Geometry: final body of the model. Coordinates: model frame, mm. Coordinates: 2 decimals unless noted, no trailing zeros. Order: outer loops, then holes, each group sorted by start corner. A loop starts at its lowest first (then second) coordinate and runs counter-clockwise, first axis right, second up. Notation, with made-up numbers: (64, -35.75) - (110, -35.75) arc R17 cw to (110, -16.75) - close; hole circle Ø8 at (-17, -18.5). An arc over 180 degrees is marked (long way). Use a Markdown table: item, result. Add a question column.
```python
from build123d import *

# Parameters (mm, degrees)
SKETCH_1_R          = 37.5
SKETCH_1_R_2        = 32.5
EXTRUDE_1_DEPTH     = 50
SKETCH_2_R          = 92.5
SKETCH_2_R_2        = 37.5
SKETCH_2_R_3        = 9
EXTRUDE_2_DEPTH     = 20
SKETCH_3_R          = 37.5
EXTRUDE_3_DEPTH     = 20
SKETCH_4_R          = 32.5
CUT_EXTRUDE_1_DEPTH = 141.044635742


with BuildPart() as part:
    # Sketch 1 → Extrude 1 (new body)
    with BuildSketch(Plane(origin=(0, 0, 0), x_dir=(1, 0, 0), z_dir=(0, 1, 0))):
        with Locations(Location((0, 0, 0), (0, 0, 270))):
            Circle(SKETCH_1_R)
        with Locations(Location((0, 0, 0), (0, 0, 270))):
            Circle(SKETCH_1_R_2, mode=Mode.SUBTRACT)
    extrude(amount=EXTRUDE_1_DEPTH)



with BuildPart() as body_2:
    # Sketch 2 → Extrude 2 (new body)
    with BuildSketch(Plane(origin=(0, 50, 0), x_dir=(1, 0, 0), z_dir=(0, 1, 0))):
        with Locations(Location((0, 0, 0), (0, 0, 270))):
            Circle(SKETCH_2_R)
        with Locations(Location((0, 0, 0), (0, 0, 270))):
            Circle(SKETCH_2_R_2, mode=Mode.SUBTRACT)
        with Locations(Location((-72.5, 0, 0), (0, 0, 270))):
            Circle(SKETCH_2_R_3, mode=Mode.SUBTRACT)
        with Locations(Location((0, 72.5, 0), (0, 0, 270))):
            Circle(SKETCH_2_R_3, mode=Mode.SUBTRACT)
        with Locations(Location((72.5, 0, 0), (0, 0, 270))):
            Circle(SKETCH_2_R_3, mode=Mode.SUBTRACT)
        with Locations(Location((0, -72.5, 0), (0, 0, 270))):
            Circle(SKETCH_2_R_3, mode=Mode.SUBTRACT)
    extrude(amount=EXTRUDE_2_DEPTH)


with BuildPart() as part_1:
    add(part.part)

    add(body_2.part)  # Extrude 3 merges body 2
    # Sketch 3 → Extrude 3 (add)
    with BuildSketch(Plane(origin=(0, 50, 0), x_dir=(1, 0, 0), z_dir=(0, 1, 0))):
        with Locations(Location((0, 0, 0), (0, 0, 270))):
            Circle(SKETCH_3_R)
    extrude(amount=EXTRUDE_3_DEPTH)

    # Sketch 4 → Cut-Extrude 1 (cut, through all)
    with BuildSketch(Plane.XZ.offset(-50)):
        with Locations(Location((0, 0, 0), (0, 0, 270))):
            Circle(SKETCH_4_R)
    extrude(amount=-CUT_EXTRUDE_1_DEPTH, mode=Mode.SUBTRACT)


solid = part_1.part
```
1) Draft query along X for faces 1 (the face through (2.703, 59.86, 81.084)), 2 (the face through (-22.818, 24.65, -29.759)), 3 (the face through (1, 50, 40)). Return one class per face: pulls with the +X half, pulls with the -X half, needs draft (parallel to the pull), parting line crosses it, or undercut.
2) Section B-B (z = 0). Return loops of the section in (x, y), then the cut area to 3 significant figures.
3) Section D-D (z = -29). Return loops of the section in (x, y).
4) Section C-C (y = 63). Return loops of the section in (x, z), then the cut area to 3 significant figures.
5) Pin query (flat end, axial travel): pin 1 (6 mm diameter, centred on x = -8.5, y = 45.5, fed in from -Z); pin 2 (1 mm diameter, centred on y = 21.5, z = 13.5, fed in from +X); pin 3 (1 mm diameter, centred on y = 11.5, z = 20, fed in from +X). Return the tip coordinate at first contact, or that it passes through.
6) Section A-A (x = 0). Return loops of the section in (y, z), then the cut area to 3 significant figures.
7) Ray query, line 1 along X through (y, z) = (56.25, 0); line 2 along X through (y, z) = (42, -1); line 3 along Y through (x, z) = (34.5, -35). Return the intervals inside material, ascending.
Values follow:
| question | item | result |
|---|---|---|
| 1 | face 1 | undercut |
| 1 | face 2 | parting line crosses it |
| 1 | face 3 | needs draft |
| 2 | outline | (-92.5, 50) - (-81.5, 50) - (-81.5, 70) - (-92.5, 70) - close; (-63.5, 50) - (-37.5, 50) - (-37.5, 0) - (-32.5, 0) - (-32.5, 70) - (-63.5, 70) - close; (32.5, 0) - (37.5, 0) - (37.5, 50) - (63.5, 50) - (63.5, 70) - (32.5, 70) - close; (81.5, 50) - (92.5, 50) - (92.5, 70) - (81.5, 70) - close |
| 2 | area | 2,180 mm² |
| 3 | outline | (-87.84, 50) - (-23.77, 50) - (-23.77, 0) - (-14.67, 0) - (-14.67, 70) - (-87.84, 70) - close; (14.67, 0) - (23.77, 0) - (23.77, 50) - (87.84, 50) - (87.84, 70) - (14.67, 70) - close |
| 4 | outline | circle Ø185 at (0, 0); hole circle Ø18 at (-72.5, 0); hole circle Ø65 at (0, 0); hole circle Ø18 at (0, -72.5); hole circle Ø18 at (0, 72.5); hole circle Ø18 at (72.5, 0) |
| 4 | area | 22,500 mm² |
| 5 | pin 1 | stops at z = -37.09 |
| 5 | pin 2 | stops at x = 35.17 |
| 5 | pin 3 | stops at x = 32.03 |
| 6 | outline | (0, -37.5) - (50, -37.5) - (50, -63.5) - (70, -63.5) - (70, -32.5) - (0, -32.5) - close; (0, 32.5) - (70, 32.5) - (70, 63.5) - (50, 63.5) - (50, 37.5) - (0, 37.5) - close; (50, -92.5) - (70, -92.5) - (70, -81.5) - (50, -81.5) - close; (50, 81.5) - (70, 81.5) - (70, 92.5) - (50, 92.5) - close |
| 6 | area | 2,180 mm² |
| 7 | line 1 | x = -92.5 to -81.5, -63.5 to -32.5, 32.5 to 63.5, 81.5 to 92.5 |
| 7 | line 2 | x = -37.49 to -32.48, 32.48 to 37.49 |
| 7 | line 3 | y = 50 to 70 |
